Geometry check sheet. Reference: the model listing, model coordinates, mm. A direction names the side the tool comes from. Give positions to 0.01 mm unless a question says otherwise; leave off trailing zeros. Loops run counter-clockwise (first coordinate to the right, second up) from the corner with the lowest first, then second, coordinate; pieces in that order, holes last. Notation, with made-up numbers: (5.5, -28.5) - (22.5, -28.5) arc R27 cw to (22.5, 7.5) - close; hole circle Ø10 at (33, 49). An arc over 180 degrees is marked (long way). Write item = value, one per line. Start each with the question number.
from build123d import *

# Parameters (mm, degrees)
CUT_EXTRUDE_1_DEPTH = 2.4


with BuildPart() as part:
    # 草图1 → Revolve 665 (revolve)
    with BuildSketch(Plane.XY, mode=Mode.PRIVATE) as revolve_665_sk:
        with BuildLine():
            Line((0, 0), (0, 7.383434901))
            ThreePointArc((0, 7.383434901), (0.026272266, 7.450993922), (0.091284426, 7.483054371))
            Line((0.091284426, 7.483054371), (6, 8))
            Line((6, 8), (6, 5.2))
            ThreePointArc((6, 5.2), (6.117157288, 4.917157288), (6.4, 4.8))
            Line((6.4, 4.8), (8.653589838, 4.8))
            Line((8.653589838, 4.8), (9, 5))
            Line((9, 5), (26, 5))
            Line((26, 5), (26, 0))
            Line((26, 0), (0, 0))
        make_face()
    revolve(revolve_665_sk.sketch.rotate(Axis((0, 0, 0), (1, 0, 0)), 90), axis=Axis((0, 0, 0), (1, 0, 0)))

    # 草图2 → 切除-拉伸1 (cut)
    with BuildSketch(Plane.ZY):
        with BuildLine():
            Line((1.25, 7.901740315), (1.25, -7.901740315))
            ThreePointArc((1.25, -7.901740315), (0, -8), (-1.25, -7.901740315))
            Line((-1.25, -7.901740315), (-1.25, 7.901740315))
            ThreePointArc((-1.25, 7.901740315), (0, 8), (1.25, 7.901740315))
        make_face()
    extrude(amount=-CUT_EXTRUDE_1_DEPTH, mode=Mode.SUBTRACT)

    # 草图3 → 切除-旋转1 (revolve, cut)
    with BuildSketch(Plane(origin=(0, 0, 0), x_dir=(1, 0, 0), z_dir=(0, 1, 0)), mode=Mode.PRIVATE) as cut_revolve_1_sk:
        Polygon((25.250022, 5), (26.749978, 5), (26, 3.701), align=None)
    revolve(cut_revolve_1_sk.sketch.rotate(Axis((0, 0, 0), (1, 0, 0)), 180), axis=Axis((0, 0, 0), (1, 0, 0)), mode=Mode.SUBTRACT)


solid = part.part
1) Material ranges on line 1 along X through (y, z) = (3, 5.5); line 2 along Y through (x, z) = (12.5, 0); line 3 along Y through (x, z) = (10, -1.25), recorded low to high.
2) Gauge pin test, flat ends, axial feed: P1, Ø2.5, axis at x = 1, y = -0.5, coming from the +Z side; P2, Ø1, axis at x = 5, z = 2, coming from the +Y side; P3, Ø1.2, axis at x = 1, y = 3.5, coming from the -Z side. Record the tip position at first contact, or that the pin passes through.
3) Cross-section at B-B on y = 0. Enter the section's corners in (x, z).
4) Release check for a two-part mould opening along X. For faces 1 (the face through (7.54, -4.05, 2.58)), 2 (the face through (1, 0, -1.25)), 3 (the face through (26, 0, 0)) record: pulls with the +X half, pulls with the -X half, needs draft (parallel to the pull), parting line crosses it, or undercut.
5) Cross-section at D-D on x = 16.75. Enter the section's corners in (y, z), and give its area (3 significant figures).
6) Cross-section at C-C on x = 6.75. Enter the section's corners in (y, z), and give its area (3 significant figures).
7) Cross-section at A-A on z = 0. Enter the section's corners in (x, y), and give its area (3 significant figures).
8) Tool access check on faces 4 (the face through (6, 5, 2)), 5 (the face through (1, 0, 1.25)), 6 (the face through (0, 0, -4)). Record the directions out of +Z, -Z, +X, -X, +Y, -Y that give a thin tool (end or side, any length) a straight path to the whole face; none if there is none.
Checked values:
q1.line_1 = 0 to 6
q1.line_2 = -5 to 5
q1.line_3 = -4.84 to 4.84
q2.P1 = 7.67
q2.P2 = 7.78
q2.P3 = -6.99
q3.outline = (0, -7.38) arc R0.1 ccw to (0.09, -7.48) - (6, -8) - (6, -5.2) arc R0.4 cw to (6.4, -4.8) - (8.65, -4.8) - (9, -5) - (25.25, -5) - (26, -3.7) - (26, 3.7) - (25.25, 5) - (9, 5) - (8.65, 4.8) - (6.4, 4.8) arc R0.4 cw to (6, 5.2) - (6, 8) - (0.09, 7.48) arc R0.1 ccw to (0, 7.38) - (0, 1.25) - (2.4, 1.25) - (2.4, -1.25) - (0, -1.25) - close
q4.face_1 = undercut
q4.face_2 = needs draft
q4.face_3 = pulls with the +X half
q5.outline = circle Ø10 at (0, 0)
q5.area = 78.5 mm²
q6.outline = circle Ø9.6 at (0, 0)
q6.area = 72.4 mm²
q7.outline = (2.4, -7.69) - (6, -8) - (6, -5.2) arc R0.4 cw to (6.4, -4.8) - (8.65, -4.8) - (9, -5) - (25.25, -5) - (26, -3.7) - (26, 3.7) - (25.25, 5) - (9, 5) - (8.65, 4.8) - (6.4, 4.8) arc R0.4 cw to (6, 5.2) - (6, 8) - (2.4, 7.69) - close
q7.area = 254 mm²
q8.face_4 = +X
q8.face_5 = -X, +Y, -Y
q8.face_6 = +Z, -Z, -X, +Y, -Y
